Check sheet for the drawn part. Datum: minimum x, y, z corner. Units: mm. Give positions to 0.01 mm unless a question says otherwise; leave off trailing zeros. Write each loop counter-clockwise with the first axis right and the second up, starting at its lowest first coordinate (ties: lowest second). Pieces come first, ordered by that corner, then holes.
(1) Thickness scan on line 1 along Y through (x, z) = (50, 12); line 2 along X through (y, z) = (30.5, 4); line 3 along Y through (x, z) = (62, 14.5). Record the ranges inside material, lowest first.
(2) Cross-section at A-A (y = 215). Record the boundary of the cut face in (x, z), and give its area (3 significant figures).
(3) Mould release check, pull along Y, two halves, no side actions. Record for the marked faces 1, 2, 3 and 4: +Y half, -Y half, draft (parallel to the pull), parting line (faces both ways), or undercut.
(4) Cross-section at D-D (z = 7). Record the boundary of the cut face in (x, y).
(5) Depth check by flat-ended pin: P1, Ø6, axis at y = 107, z = 13, coming from the -X side. Enter the tip coordinate at first touch or a pass-through.
(6) Cross-section at C-C (y = 30). Record the boundary of the cut face in (x, z).
(7) Cross-section at B-B (x = 50). Record the boundary of the cut face in (y, z), and give its area (3 significant figures).
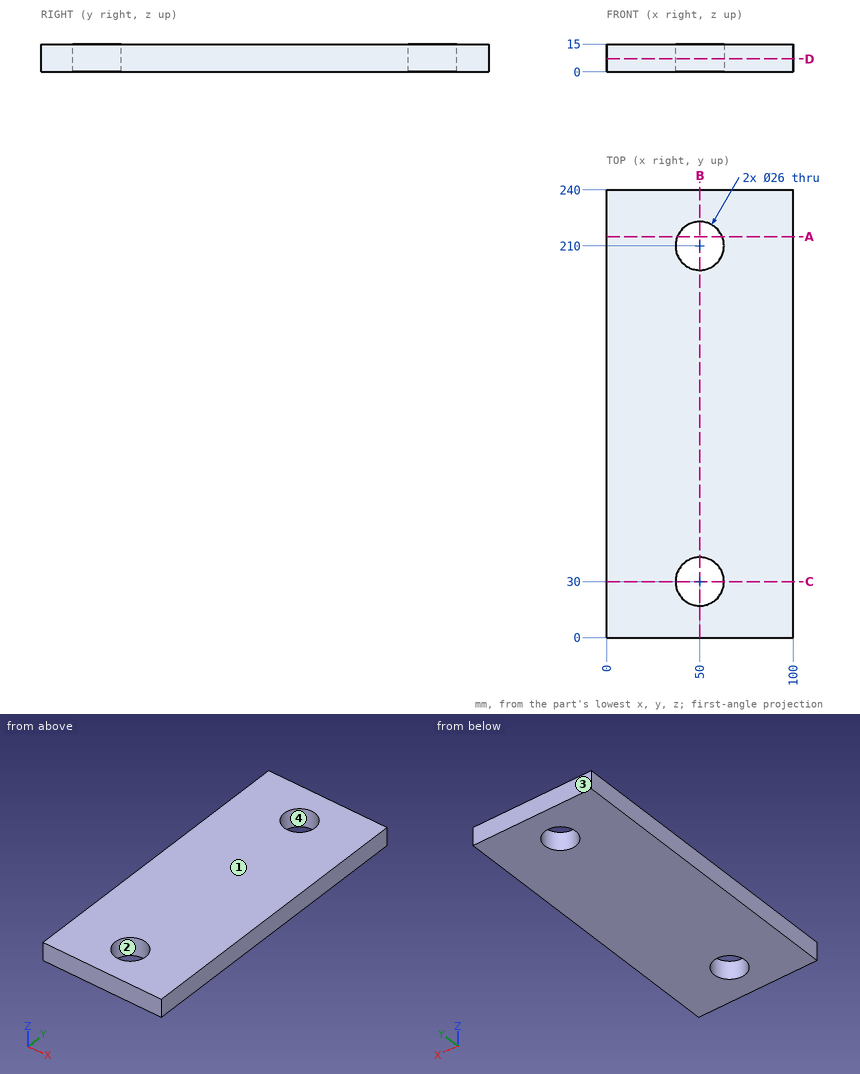
Reply:
1. line 1: y = 0 to 17, 43 to 197, 223 to 240
1. line 2: x = 0 to 37.01, 62.99 to 100
1. line 3: y = 0 to 25, 35 to 205, 215 to 240
2. outline: (0, 0) - (38, 0) - (38, 15) - (0, 15) - close; (62, 0) - (100, 0) - (100, 15) - (62, 15) - close
2. area: 1,140 mm2
3. face 1: draft
3. face 2: undercut
3. face 3: +Y half
3. face 4: undercut
4. outline: (0, 0) - (100, 0) - (100, 240) - (0, 240) - close; hole circle Ø26 at (50, 30); hole circle Ø26 at (50, 210)
5. P1: stops at x = 0
6. outline: (0, 0) - (37, 0) - (37, 15) - (0, 15) - close; (63, 0) - (100, 0) - (100, 15) - (63, 15) - close
7. outline: (0, 0) - (17, 0) - (17, 15) - (0, 15) - close; (43, 0) - (197, 0) - (197, 15) - (43, 15) - close; (223, 0) - (240, 0) - (240, 15) - (223, 15) - close
7. area: 2,820 mm2
